Geometry check sheet. Reference: the model listing, model coordinates, mm. A direction names the side the tool comes from. Give positions to 0.01 mm unless a question says otherwise; leave off trailing zeros. Order: outer loops, then holes, each group sorted by start corner. A loop starts at its lowest first (then second) coordinate and runs counter-clockwise, first axis right, second up.
from build123d import *

# Parameters (mm, degrees)
BASE_PLATE_SKETCH_W        = 150
BASE_PLATE_SKETCH_H        = 90
BASE_PLATE_150X90X15_DEPTH = 15
BOSS_TUBE_SKETCH_R         = 33
BOSS_TUBE_SKETCH_R_2       = 21
BOSS_TUBE_66_DEPTH         = 50
OVAL_FLANGE_SKETCH_RX      = 60
OVAL_FLANGE_SKETCH_RY      = 36
OVAL_FLANGE_SKETCH_R       = 21
OVAL_FLANGE_120X72_DEPTH   = 15
BASE_BORE_SKETCH_R         = 16.5
BASE_BORE_33_DEPTH         = 15
FLANGE_BOLT_HOLE_SKETCH_R  = 6
FLANGE_BOLT_HOLE_DEPTH     = 15


with BuildPart() as part:
    # Base Plate Sketch → Base Plate 150x90x15 (new body)
    with BuildSketch(Plane(origin=(0, 0, 0), x_dir=(1, 0, 0), z_dir=(0, 1, 0))):
        Rectangle(BASE_PLATE_SKETCH_W, BASE_PLATE_SKETCH_H)
    extrude(amount=BASE_PLATE_150X90X15_DEPTH)

    # Boss Tube Sketch → Boss Tube Ø66 (add)
    with BuildSketch(Plane(origin=(0, 15, 0), x_dir=(1, 0, 0), z_dir=(0, 1, 0))):
        with Locations(Location((0, 0, 0), (0, 0, 90))):
            Circle(BOSS_TUBE_SKETCH_R)
        with Locations(Location((0, 0, 0), (0, 0, 270))):
            Circle(BOSS_TUBE_SKETCH_R_2, mode=Mode.SUBTRACT)
    extrude(amount=BOSS_TUBE_66_DEPTH)

    # Oval Flange Sketch → Oval Flange 120x72 (add)
    with BuildSketch(Plane(origin=(0, 65, 0), x_dir=(1, 0, 0), z_dir=(0, 1, 0))):
        with Locations((0, 0)):
            Ellipse(OVAL_FLANGE_SKETCH_RX, OVAL_FLANGE_SKETCH_RY)
        with Locations(Location((0, 0, 0), (0, 0, 270))):
            Circle(OVAL_FLANGE_SKETCH_R, mode=Mode.SUBTRACT)
    extrude(amount=OVAL_FLANGE_120X72_DEPTH)

    # Base Bore Sketch → Base Bore Ø33 (cut)
    with BuildSketch(Plane(origin=(0, 15, 0), x_dir=(1, 0, 0), z_dir=(0, 1, 0))):
        with Locations(Location((0, 0, 0), (0, 0, 270))):
            Circle(BASE_BORE_SKETCH_R)
    extrude(amount=-BASE_BORE_33_DEPTH, mode=Mode.SUBTRACT)

    # Flange Bolt Hole Sketch → Flange Bolt Hole (cut)
    with BuildSketch(Plane(origin=(0, 80, 0), x_dir=(1, 0, 0), z_dir=(0, 1, 0))):
        with Locations(Location((-41.995846121, 0, 0), (0, 0, 270))):
            Circle(FLANGE_BOLT_HOLE_SKETCH_R)
        with Locations(Location((41.995846121, 0, 0), (0, 0, 90))):
            Circle(FLANGE_BOLT_HOLE_SKETCH_R)
    extrude(amount=-FLANGE_BOLT_HOLE_DEPTH, mode=Mode.SUBTRACT)


solid = part.part
Item 1: Gauge pin test, flat ends, axial feed: pin 1 (4 mm diameter, centred on y = 47, z = -7, fed in from +X); pin 2 (7 mm diameter, centred on x = 42, z = 0, fed in from +Y); pin 3 (3 mm diameter, centred on x = 55.5, y = 68, fed in from +Z). Record the tip position at first contact, or that the pin passes through.
Reported:
pin 1: stops at x = 32.62
pin 2: stops at y = 15
pin 3: stops at z = 15.69
Item 2: Sectioned sample at A-A (z = 0). Give the number of separate pieces and of enclosed holes in the cut face, and give its area (4 significant figures).
Reported:
separate pieces: 4
enclosed holes: 0
area: 3,765 mm2
Item 3: Draft check along X on faces 1 (the flat face through (75, 7, 1)), 2 (the flat face through (-34, 15, -1)), 3 (the cylindrical face through (6.31, 47.04, 20.03)). Enter one of: released by +X, released by -X, zero draft, split by the parting line, or undercut.
Reported:
face 1: released by +X
face 2: zero draft
face 3: undercut
Item 4: Sectioned sample at C-C (z = 40). Enter the section's corners in (x, y).
Reported:
outline: (-75, 0) - (75, 0) - (75, 15) - (-75, 15) - close
Item 5: Set-up check for faces 4 (the flat face through (-1, 7, 45)), 5 (the cylindrical face through (32.215, 39.65, 7.154)), 6 (the flat face through (-13, 15, 11)): record each of +Z, -Z, +X, -X, +Y, -Y from which the full face is reachable in a straight line by a thin tool's end or side.
Reported:
face 4: +Z, +X, -X, +Y, -Y
face 5: none
face 6: +Y
Item 6: Scan lines: L1, parallel to X at y = 56, z = 0; L2, parallel to X at y = 3, z = 0; L3, parallel to Y at x = 59.5, z = 1.5. Record each from-to range of solid material in increasing order.
Reported:
L1: x = -33 to -21, 21 to 33
L2: x = -75 to -16.5, 16.5 to 75
L3: y = 0 to 15, 65 to 80
